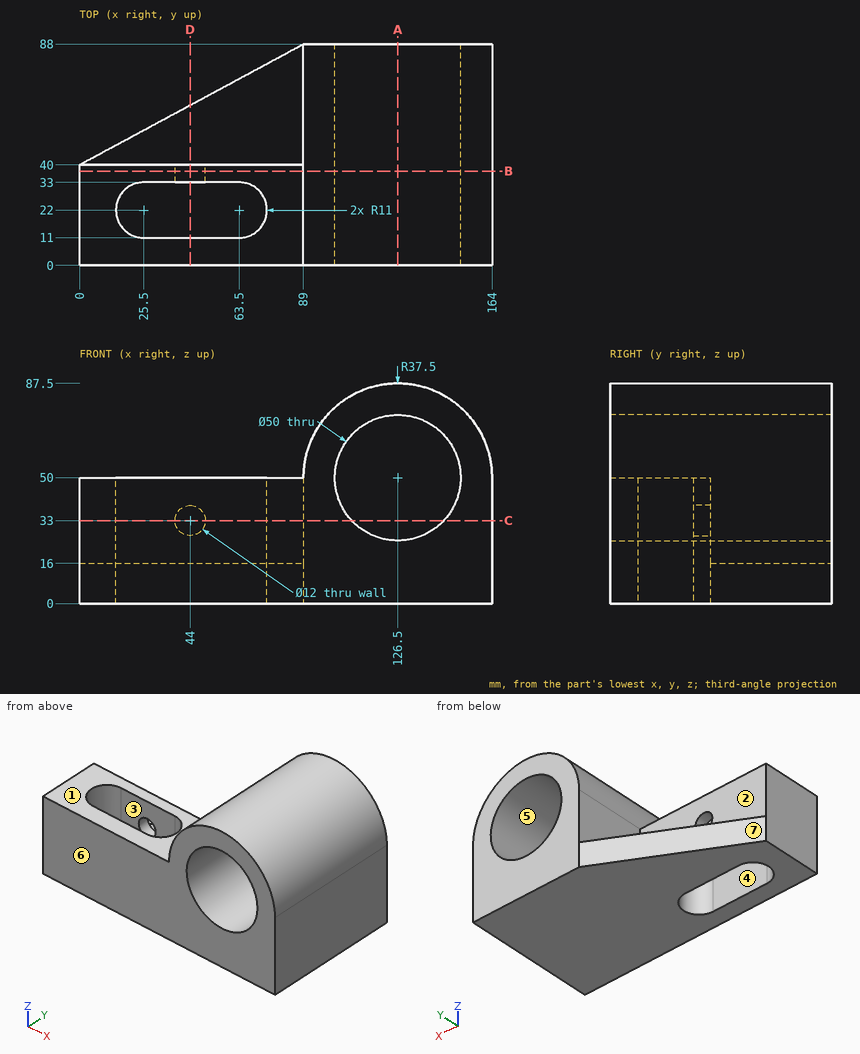
Geometry check sheet. Reference: drawing and pictorial views, mm from the part's lowest x, y, z. A direction names the side the tool comes from. Round coordinates to 2 decimals unless told otherwise and drop trailing zeros. Order: outer loops, then holes, each group sorted by start corner. A loop starts at its lowest first (then second) coordinate and runs counter-clockwise, first axis right, second up. Notation, with made-up numbers: M -37.75,39.25 L -1.75,39.25 A30 ccw -1.75,78.25 Z; hole C -9,-24.5 d8. An arc over 180 degrees is marked long. Answer in a Markdown table with one row per item.
(1) Sectioned sample at C-C, the plane z = 33. Record the cut outline in (x, y).
Responses:
| item | result |
|---|---|
| outline | M 0,0 L 108.17,0 L 108.17,88 L 89,88 L 89,40 L 50,40 L 50,33 L 63.5,33 A11 cw 63.5,11 L 25.5,11 A11 cw 25.5,33 L 38,33 L 38,40 L 0,40 Z; M 144.83,0 L 164,0 L 164,88 L 144.83,88 Z |
(2) Draft check along X on the marked faces 4, 5, 6 and 7. Enter one of: released by +X, released by -X, zero draft, split by the parting line, or undercut.
Responses:
| item | result |
|---|---|
| face 4 | undercut |
| face 5 | undercut |
| face 6 | zero draft |
| face 7 | released by -X |
(3) Sectioned sample at A-A, the plane x = 126.5. Record the cut outline in (y, z), and give its area (3 significant figures).
Responses:
| item | result |
|---|---|
| outline | M 0,0 L 88,0 L 88,25 L 0,25 Z; M 0,75 L 88,75 L 88,87.5 L 0,87.5 Z |
| area | 3,300 mm² |
(4) Tool access check on the marked faces 1, 2 and 3. Record the directions out of +Z, -Z, +X, -X, +Y, -Y that give a thin tool (end or side, any length) a straight path to the whole face; none if there is none.
Responses:
| item | result |
|---|---|
| face 1 | +Z, -X, +Y, -Y |
| face 2 | +Z, -X, +Y |
| face 3 | +Z, -Z |
(5) Scan lines: probe 1 along Y at (x, z) = (34.5, 24.5); probe 2 along X at (y, z) = (47, 50); probe 3 along Y at (x, z) = (87, 39). Record each from-to range of solid material in increasing order. Write a range as from..to.
Responses:
| item | result |
|---|---|
| probe 1 | y = 0..11, 33..40 |
| probe 2 | x = 89..101.5, 151.5..164 |
| probe 3 | y = 0..40 |
(6) Go/stop test with flat-tipped pins: P1, Ø17, axis at x = 54.5, z = 41, coming from the +Y side; P2, Ø3, axis at y = 63.5, z = 49.5, coming from the -X side; P3, Ø2, axis at y = 79, z = 53.5, coming from the +X side. Record where each tip stops, or that it passes through.
Responses:
| item | result |
|---|---|
| P1 | stops at y = 40 |
| P2 | stops at x = 89 |
| P3 | stops at x = 163.92 |
(7) Sectioned sample at B-B, the plane y = 37.5. Record the cut outline in (x, z).
Responses:
| item | result |
|---|---|
| outline | M 0,0 L 164,0 L 164,50 A37.5 ccw 89,50 L 0,50 Z; hole C 44,33 d12; hole C 126.5,50 d50 |
(8) Sectioned sample at D-D, the plane x = 44. Record the cut outline in (y, z).
Responses:
| item | result |
|---|---|
| outline | M 0,0 L 11,0 L 11,50 L 0,50 Z; M 33,0 L 63.73,0 L 63.73,16 L 40,16 L 40,27 L 33,27 Z; M 33,39 L 40,39 L 40,50 L 33,50 Z |
